Input: dimensioned drawing with shaded views. Units: mm. Origin: part minimum x, y, z. A direction names the side the tool comes from. Round coordinates to 2 decimals unless told otherwise and drop trailing zeros. Write each loop counter-clockwise with the first axis right and the second up, starting at its lowest first coordinate (ties: lowest second). Pieces come first, ordered by that corner, then holes. Notation, with made-up numbers: M 86,59.5 L 114,59.5 A12 ccw 114,63.5 Z; hole C -26,-5 d5. An arc over 180 degrees is marked long. Put each result on its own line as item: value. Start each with the question number.
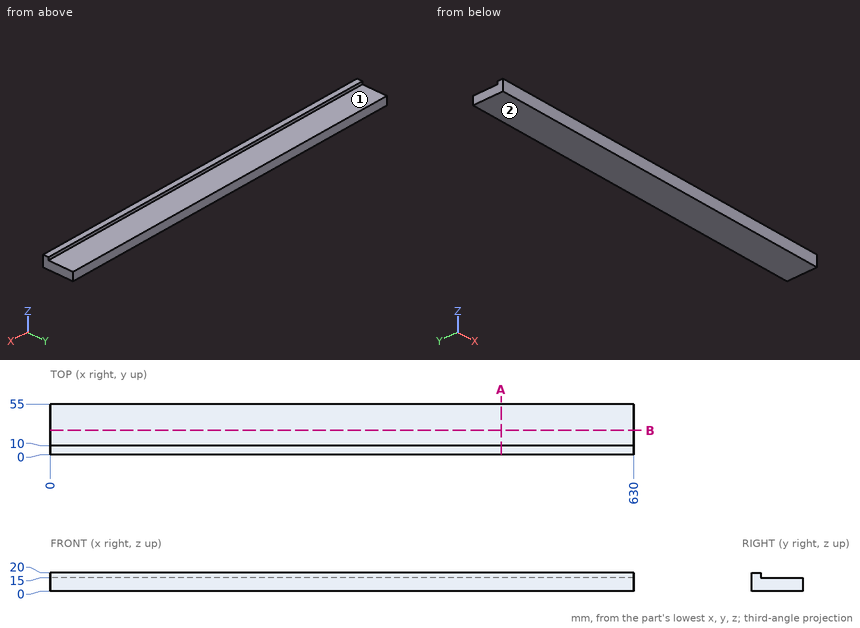
1) Section A-A, the plane x = 487. Output: boundary loops of the cut face in (y, z), and give its area (3 significant figures).
2) Access query for the marked faces 1 and 2. Directions: +Z, -Z, +X, -X, +Y, -Y. A direction counts if a zero-diameter tool reaches every point of the face in a straight line with its end or side. Return the directions, or none.
3) Section B-B, the plane y = 26.5. Output: boundary loops of the cut face in (x, z).
4) Ray query, probe 1 along Z at (x, y) = (595.5, 40.5); probe 2 along Y at (x, z) = (204.5, 18.75). Return the intervals inside material, ascending.
5) First-contact query: pin 1 (10 mm diameter, centred on x = 297, y = 16.5, fed in from -Z); pin 2 (10 mm diameter, centred on x = 106, y = 31.5, fed in from +Z); pin 3 (4 mm diameter, centred on x = 231.5, z = 18, fed in from +Y). Flat tips, straight axial feed; report the tip coordinate or a pass-through.
Solved:
1. outline: M 0,0 L 55,0 L 55,15 L 10,15 L 10,20 L 0,20 Z
1. area: 875 mm2
2. face 1: +Z, +X, -X, +Y
2. face 2: -Z, +X, -X, +Y, -Y
3. outline: M 0,0 L 630,0 L 630,15 L 0,15 Z
4. probe 1: z = 0 to 15
4. probe 2: y = 0 to 10
5. pin 1: stops at z = 0
5. pin 2: stops at z = 15
5. pin 3: stops at y = 10
